```python
from build123d import *

# Parameters (mm, degrees)
EXTRUDE_1_DEPTH = 34


with BuildPart() as part:
    # 草图2 → 拉伸-薄壁1 (new, symmetric)
    with BuildSketch(Plane(origin=(290.969985959, -860.871008049, 2246.011610274), x_dir=(-0.12461162955889699, -0.382773527459934, 0.9153995676504089), z_dir=(0.8091108722091485, 0.49479707812616053, 0.3170417132661968))):
        with BuildLine():
            Line((0, 712.5), (0, -209.427913233))
            ThreePointArc((0, -209.427913233), (-62, -271.427913233), (-124, -209.427913233))
            Line((-124, -209.427913233), (-124, 297.758706857))
            Line((-124, 297.758706857), (-89, 297.758706857))
            Line((-89, 297.758706857), (-89, -209.427913233))
            ThreePointArc((-89, -209.427913233), (-62, -236.427913233), (-35, -209.427913233))
            Line((-35, -209.427913233), (-35, 712.5))
            Line((-35, 712.5), (0, 712.5))
        make_face()
    extrude(amount=EXTRUDE_1_DEPTH, both=True)


solid = part.part
```
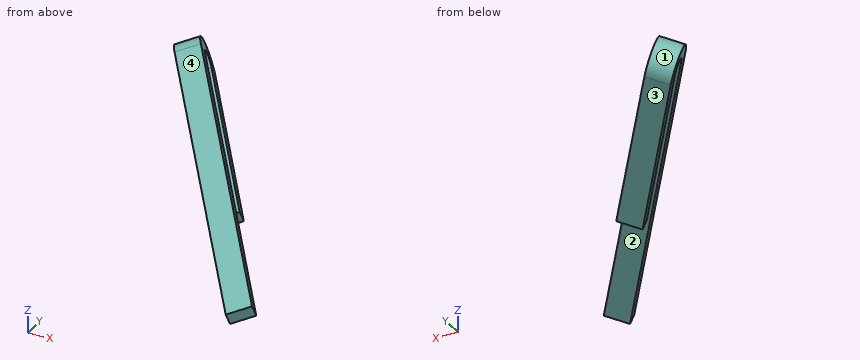
Verification items for the finished model (mm, model axes). Face numbers are marked on the shaded views. Give positions to 0.01 mm unless a question says otherwise; leave off trailing zeros. Order: outer loops, then holes, each group sorted by start corner. A loop starts at its lowest first (then second) coordinate and runs counter-clockwise, first axis right, second up. Notation, with made-up numbers: M 55.25,-33.5 L 95.25,-33.5 A15 ccw 95.25,-18.5 Z; hole C 8.5,-27.5 d8. An arc over 180 degrees is marked long. Return JSON: item names as keys, results as strings. Group by question number.
1) Go/stop test with flat-tipped pins: pin 1 Ø1 at (x, z) = (252.5, 2147.5) entering from -Y; pin 2 Ø1 at (x, z) = (412, 2105.5) entering from -Y; pin 3 Ø2 at (y, z) = (-1286, 2069) entering from -X. Record where each tip stops, or that it passes through.
2) Mould release check, pull along Z, two halves, no side actions. Record for the marked faces 1, 2, 3 and 4: pulls with the +Z half, pulls with the -Z half, needs draft (parallel to the pull), parting line crosses it, or undercut.
3) Section check C-C on x = 534.5. Record the cut outline in (y, z), and give its area (3 significant figures).
4) Section check D-D on y = -1100.5. Record the cut outline in (x, z).
5) Section check B-B on y = -833.5. Record the cut outline in (x, z), and give its area (3 significant figures).
6) Section check A-A on z = 2112. Record the cut outline in (x, y), and give its area (3 significant figures).
7) Scan lines: line 1 (Y direction, x = 428, z = 2112.5); line 2 (Y direction, x = 643, z = 2065.5); line 3 (Z direction, x = 511, y = -1135.5). Record each from-to range of solid material in increasing order.
Answer block:
{
 "1": {"pin 1": "stops at y = -804.44", "pin 2": "stops at y = -1005", "pin 3": "stops at x = 577.56"},
 "2": {"face 1": "parting line crosses it", "face 2": "undercut", "face 3": "pulls with the -Z half", "face 4": "pulls with the +Z half"},
 "3": {"outline": "M -1245.9,2118.16 L -1226.58,2088.01 L -1118.19,2133.33 L -1137.51,2163.49 Z", "area": "4,140 mm^2"},
 "4": {"outline": "M 427.47,2164.39 L 441.69,2128.09 L 521.48,2138.96 L 507.26,2175.25 Z"},
 "5": {"outline": "M 230.93,2249.28 L 245.15,2212.98 L 324.94,2223.85 L 310.72,2260.14 Z; M 267.1,2156.98 L 281.32,2120.68 L 361.11,2131.54 L 346.88,2167.84 Z", "area": "6,100 mm^2"},
 "6": {"outline": "M 301.42,-860.81 L 371.24,-974.98 L 476.17,-1009.14 L 406.36,-894.97 Z; M 478.96,-1151.12 L 548.77,-1265.29 L 653.71,-1299.45 L 583.89,-1185.28 Z", "area": "19,200 mm^2"},
 "7": {"line 1": "y = -992.26 to -930.68", "line 2": "y = -1389.58 to -1315.73", "line 3": "z = 2122.89 to 2161.13"}
}
